Verification items for the finished model (mm, model axes). A direction names the side the tool comes from. Give positions to 0.01 mm unless a question says otherwise; leave off trailing zeros. Loops run counter-clockwise (first coordinate to the right, second up) from the corner with the lowest first, then second, coordinate; pieces in that order, holes last. Notation, with made-up numbers: (-7.75, 53.25) - (3.25, 53.25) arc R23 cw to (3.25, 81.25) - close; hole circle Ø8 at (64.25, 88.25). An arc over 180 degrees is marked (long way). Answer in a Markdown table with one row per item.
```python
from build123d import *

# Parameters (mm, degrees)
SKETCH1_W              = 2000
SKETCH1_H              = 600
BOSS_EXTRUDE1_DEPTH    = 20
SKETCH2_W              = 250
SKETCH2_H              = 360
CUT_EXTRUDE1_DEPTH     = 1045.222198577
SKETCH3_W              = 60
SKETCH3_H              = 50
BOSS_EXTRUDE2_DEPTH    = 51
SKETCH4_W              = 60
SKETCH4_H              = 12
CUT_EXTRUDE2_DEPTH     = 40
FILLET1_R              = 12
SKETCH5_R              = 10
CUT_EXTRUDE3_DEPTH     = 1060.885489098
LPATTERN1_COUNT        = 2
LPATTERN1_PITCH        = 120
FILLET1_OF_LPATTERN1_R = 12


with BuildPart() as part:
    # Sketch1 → Boss-Extrude1 (new body)
    with BuildSketch(Plane.XY):
        Rectangle(SKETCH1_W, SKETCH1_H)
    extrude(amount=BOSS_EXTRUDE1_DEPTH)

    # Sketch2 → Cut-Extrude1 (cut, through all)
    with BuildSketch(Plane(origin=(0, 0, 0), x_dir=(-1, 0, 0), z_dir=(0, 0, -1))):
        with Locations((-700, 0)):
            Rectangle(SKETCH2_W, SKETCH2_H)
    extrude(amount=-CUT_EXTRUDE1_DEPTH, mode=Mode.SUBTRACT)

    # Sketch3 → Boss-Extrude2 (add)
    with BuildSketch(Plane(origin=(0, 0, 0), x_dir=(-1, 0, 0), z_dir=(0, 0, -1))):
        with Locations((-350, -22.5)):
            Rectangle(SKETCH3_W, SKETCH3_H)
    boss_extrude2 = extrude(amount=BOSS_EXTRUDE2_DEPTH)

    # Sketch4 → Cut-Extrude2 (cut)
    with BuildSketch(Plane(origin=(0, 0, -51), x_dir=(-1, 0, 0), z_dir=(0, 0, -1))):
        with Locations((-350, -23.5)):
            Rectangle(SKETCH4_W, SKETCH4_H)
    cut_extrude2 = extrude(amount=-CUT_EXTRUDE2_DEPTH, mode=Mode.SUBTRACT)

    # Fillet1
    fillet1_edges = [part.edges().sort_by_distance(p)[0] for p in [
        (380, -7.5, -51),
        (320, -38.5, -51),
        (380, -38.5, -51),
        (320, -7.5, -51),
    ]]
    fillet(fillet1_edges, radius=FILLET1_R)

    # Sketch5 → Cut-Extrude3 (cut, through all)
    with BuildSketch(Plane.XZ.offset(47.5)):
        with Locations((350, -26)):
            Circle(SKETCH5_R)
    cut_extrude3 = extrude(amount=-CUT_EXTRUDE3_DEPTH, mode=Mode.SUBTRACT)

    # LPattern1: Boss-Extrude2, Cut-Extrude2, Cut-Extrude3 ×2
    with Locations(*[(-i * LPATTERN1_PITCH, 0, 0) for i in range(1, LPATTERN1_COUNT)]):
        add(boss_extrude2)
        add(cut_extrude2, mode=Mode.SUBTRACT)
        add(cut_extrude3, mode=Mode.SUBTRACT)

    # Fillet1 of LPattern1
    fillet1_of_lpattern1_edges = [part.edges().sort_by_distance(p)[0] for p in [
        (260, -7.5, -51),
        (200, -38.5, -51),
        (260, -38.5, -51),
        (200, -7.5, -51),
    ]]
    fillet(fillet1_of_lpattern1_edges, radius=FILLET1_OF_LPATTERN1_R)


solid = part.part
```
Q1. Tool access check on faces 5 (the face through (230, 2.5, -14)), 6 (the face through (237, -29.5, -36)), 7 (the face through (-14, 4, 20)), 8 (the face through (200, -17, -19)), 9 (the face through (230, -47.5, -14)). Record the directions out of +Z, -Z, +X, -X, +Y, -Y that give a thin tool (end or side, any length) a straight path to the whole face; none if there is none.
Completed:
| item | result |
|---|---|
| face 5 | -Z, +X, -X, +Y |
| face 6 | -Z, +X, -X |
| face 7 | +Z, +X, -X, +Y, -Y |
| face 8 | -Z, -X, +Y, -Y |
| face 9 | -Z, +X, -X, -Y |
Q2. Sectioned sample at C-C (x = -795). Record the cut outline in (y, z).
Completed:
| item | result |
|---|---|
| outline | (-300, 0) - (300, 0) - (300, 20) - (-300, 20) - close |
Q3. Sectioned sample at B-B (y = 211). Record the cut outline in (x, z), and give its area (3 significant figures).
Completed:
| item | result |
|---|---|
| outline | (-1000, 0) - (1000, 0) - (1000, 20) - (-1000, 20) - close |
| area | 40,000 mm^2 |
Q4. Thickness scan on line 1 (Z direction, x = 350, y = -34.25); line 2 (X direction, y = -64, z = 5); line 3 (Z direction, x = -269, y = 220.5). Record the ranges inside material, lowest first.
Completed:
| item | result |
|---|---|
| line 1 | -51 to -36, -16 to 20 |
| line 2 | -1000 to 575, 825 to 1000 |
| line 3 | 0 to 20 |
Q5. Draft check along X on faces 1 (the face through (260, -17, -19)), 2 (the face through (350, -47.5, -14)), 3 (the face through (380, -17, -19)), 4 (the face through (320, -17, -19)). Enter one of: +X half, -X half, draft (parallel to the pull), parting line (faces both ways), or undercut.
Completed:
| item | result |
|---|---|
| face 1 | undercut |
| face 2 | draft |
| face 3 | +X half |
| face 4 | undercut |
Q6. Sectioned sample at A-A (x = 645). Record the cut outline in (y, z), and give its area (3 significant figures).
Completed:
| item | result |
|---|---|
| outline | (-300, 0) - (-180, 0) - (-180, 20) - (-300, 20) - close; (180, 0) - (300, 0) - (300, 20) - (180, 20) - close |
| area | 4,800 mm^2 |
Q7. Go/stop test with flat-tipped pins: P1, Ø18, axis at x = 230, z = -26, coming from the +Y side; P2, Ø6, axis at x = 225.5, y = -22, coming from the -Z side; P3, Ø23, axis at x = 230, z = -26, coming from the +Y side; P4, Ø3, axis at x = -770, y = -15, coming from the -Z side. Record where each tip stops, or that it passes through.
Completed:
| item | result |
|---|---|
| P1 | through |
| P2 | z = -11 |
| P3 | y = 2.5 |
| P4 | z = 0 |
